```python
from build123d import *

# Parameters (mm, degrees)
SKETCH2_R                                           = 5.25
CUT_EXTRUDE1_DEPTH                                  = 71.256672281
CUT_EXTRUDE2_REACH                                  = 63.123
HOLE_SIZE_PER_HEX_SOCKET_HEAD_CAP_SCREW_D           = 6.6
HOLE_SIZE_PER_HEX_SOCKET_HEAD_CAP_SCREW_CBORE_D     = 11
HOLE_SIZE_PER_HEX_SOCKET_HEAD_CAP_SCREW_CBORE_DEPTH = 6.8
CHAMFER1_SIZE                                       = 0.2
CHAMFER2_SIZE                                       = 0.2
CHAMFER3_SIZE                                       = 1


with BuildPart() as part:
    # Sketch1 → Revolve1 (revolve)
    with BuildSketch(Plane.XY, mode=Mode.PRIVATE) as revolve1_sk:
        Polygon((0, 0), (0, 13), (44, 13), (44, 30), (56, 30), (56, 11), (6, 11), (6, 0), align=None)
    revolve(revolve1_sk.sketch.rotate(Axis((0, 0, 0), (1, 0, 0)), 90), axis=Axis((0, 0, 0), (1, 0, 0)))

    # Sketch2 → Cut-Extrude1 (cut, through all)
    with BuildSketch(Plane.ZY):
        Circle(SKETCH2_R)
    extrude(amount=-CUT_EXTRUDE1_DEPTH, mode=Mode.SUBTRACT)

    # Sketch3 → Cut-Extrude2 (cut, up to next)
    with BuildSketch(Plane.ZY.offset(-44), mode=Mode.PRIVATE) as cut_extrude2_sk1:
        with BuildLine():
            Line((27.037011669, 13), (-27.037011669, 13))
            ThreePointArc((-27.037011669, 13), (0, 30), (27.037011669, 13))
        make_face()
    cut_extrude2_tool1 = extrude(cut_extrude2_sk1.sketch, amount=-CUT_EXTRUDE2_REACH, mode=Mode.PRIVATE) & part.part
    # Sketch3 → Cut-Extrude2 (cut, up to next)
    with BuildSketch(Plane.ZY.offset(-44), mode=Mode.PRIVATE) as cut_extrude2_sk2:
        with BuildLine():
            Line((27.037011669, -13), (-27.037011669, -13))
            ThreePointArc((-27.037011669, -13), (0, -30), (27.037011669, -13))
        make_face()
    cut_extrude2_tool2 = extrude(cut_extrude2_sk2.sketch, amount=-CUT_EXTRUDE2_REACH, mode=Mode.PRIVATE) & part.part
    add(cut_extrude2_tool1.solids().sort_by_distance((44, 19.998046, 0))[0], mode=Mode.SUBTRACT)
    add(cut_extrude2_tool2.solids().sort_by_distance((44, -19.998046, 0))[0], mode=Mode.SUBTRACT)

    # Hole size per hex socket head cap screw type 1 (through all)
    with Locations(Plane(origin=(44, -6.952882373, 21.398771617), x_dir=(0, 0, -1), z_dir=(-1, 0, 0))):
        with Locations((0, 0), (0, -13.905764746), (42.797543234, -13.905764746), (42.797543234, 0)):
            CounterBoreHole(HOLE_SIZE_PER_HEX_SOCKET_HEAD_CAP_SCREW_D / 2, HOLE_SIZE_PER_HEX_SOCKET_HEAD_CAP_SCREW_CBORE_D / 2, HOLE_SIZE_PER_HEX_SOCKET_HEAD_CAP_SCREW_CBORE_DEPTH)

    # Chamfer1
    chamfer1_edges = [part.edges().sort_by_distance(p)[0] for p in [
        (0, 0, -5.25),
        (56, 0, 30),
        (44, 0, 30),
        (56, 0, -30),
        (44, 0, -30),
        (0, 0, -13),
    ]]
    chamfer(chamfer1_edges, length=CHAMFER1_SIZE)

    # Chamfer2
    chamfer2_edges = [part.edges().sort_by_distance(p)[0] for p in [
        (56, 0, -11),
    ]]
    chamfer(chamfer2_edges, length=CHAMFER2_SIZE)

    # Chamfer3
    chamfer3_edges = [part.edges().sort_by_distance(p)[0] for p in [
        (6, 0, -5.25),
    ]]
    chamfer(chamfer3_edges, length=CHAMFER3_SIZE)


solid = part.part
```
Geometry: final body of the model. Coordinates: model frame, mm. A direction names the side the tool comes from. Give positions to 0.01 mm unless a question says otherwise; leave off trailing zeros. Loops run counter-clockwise (first coordinate to the right, second up) from the corner with the lowest first, then second, coordinate; pieces in that order, holes last. Notation, with made-up numbers: (72.25, 56.5) - (110.25, 56.5) arc R24 ccw to (110.25, 88.5) - close; hole circle Ø7 at (33, -5.5). An arc over 180 degrees is marked (long way). Answer as CSV lines item,"result". Start each with the question number.
(1) Section query C-C (x = 51.5). Output: boundary loops of the cut face in (y, z).
(2) Reachability of faces 1 (the face through (53.44, 6.81, 18.1)), 2 (the face through (44, 0, 18)), 3 (the face through (47.352, 6.711, -15.904)), 4 (the face through (30.55, 10.74, -2.38)) from +Z, -Z, +X, -X, +Y, -Y: full face, straight path, thin tool, end or side. Return the list, or none.
(3) Ray query, line 1 along Z through (x, y) = (46, 11.25); line 2 along Y through (x, z) = (3, 0); line 3 along Z through (x, y) = (53.5, -5.25). Return the intervals inside material, ascending. Write a range as [from, to].
(4) Section query B-B (x = 39.5). Output: boundary loops of the cut face in (y, z), and give its area (3 significant figures).
(5) Section query D-D (y = -8.25). Give the number of separate pieces and of enclosed holes in the cut face, and give its area (3 significant figures).
(6) Section query A-A (y = 0). Output: boundary loops of the cut face in (x, z).
(7) Mould query, pull axis Z, two halves, no side actions, for faces 5 (the face through (50, 0, -30)), 6 (the face through (22.407, 7.91, -10.316)), 7 (the face through (47.352, -7.195, -15.904)). Classes: +Z half, -Z half, draft (parallel to the pull), parting line (faces both ways), or undercut.
(8) Pin query (flat end, axial travel): P1, Ø14.5, axis at y = -6.95, z = 21.4, coming from the -X side; P2, Ø1.5, axis at x = 24.5, y = 4.5, coming from the +Z side; P3, Ø3.5, axis at y = -9, z = -21, coming from the -X side. Return the tip coordinate at first contact, or that it passes through.
Worked answers:
1,outline,"(-13, -27.04) arc R30 ccw to (13, -27.04) - (13, 27.04) arc R30 ccw to (-13, 27.04) - close; hole circle Ø22 at (0, 0); hole circle Ø6.6 at (-6.95, -21.4); hole circle Ø6.6 at (-6.95, 21.4); hole circle Ø6.6 at (6.95, -21.4); hole circle Ø6.6 at (6.95, 21.4)"
2,face 1,"+X, -X"
2,face 2,"+Z, -X"
2,face 3,"-X"
2,face 4,"+X"
3,line 1,"z = [-27.81, -24.83], [-17.97, 17.97], [24.83, 27.81]"
3,line 2,"y = [-13, -5.25], [5.25, 13]"
3,line 3,"z = [-29.54, -24.23], [-18.57, -9.67], [9.67, 18.57], [24.23, 29.54]"
4,outline,"circle Ø26 at (0, 0); hole circle Ø22 at (0, 0)"
4,area,"151 mm^2"
5,separate pieces,"3"
5,enclosed holes,"0"
5,area,"640 mm^2"
6,outline,"(0, -12.8) - (0.2, -13) - (44, -13) - (44, -29.8) - (44.2, -30) - (55.8, -30) - (56, -29.8) - (56, -11.2) - (55.8, -11) - (6, -11) - (6, -6.25) - (5, -5.25) - (0.2, -5.25) - (0, -5.45) - close; (0, 5.45) - (0.2, 5.25) - (5, 5.25) - (6, 6.25) - (6, 11) - (55.8, 11) - (56, 11.2) - (56, 29.8) - (55.8, 30) - (44.2, 30) - (44, 29.8) - (44, 13) - (0.2, 13) - (0, 12.8) - close"
7,face 5,"-Z half"
7,face 6,"parting line"
7,face 7,"undercut"
8,P1,"stops at x = 44"
8,P2,"stops at z = 12.45"
8,P3,"stops at x = 50.8"
